Source: three-view drawing plus pictorial views. Frame: mm from the lowest corner of the part. A direction names the side the tool comes from. Coordinates: 2 decimals unless noted, no trailing zeros. Order: outer loops, then holes, each group sorted by start corner. A loop starts at its lowest first (then second) coordinate and runs counter-clockwise, first axis right, second up. Notation, with made-up numbers: M 88,77 L 102,77 A22 cw 102,95 Z; hole C -2,61.5 d1. An arc over 180 degrees is marked long. One line per question, with ' | ' between items.
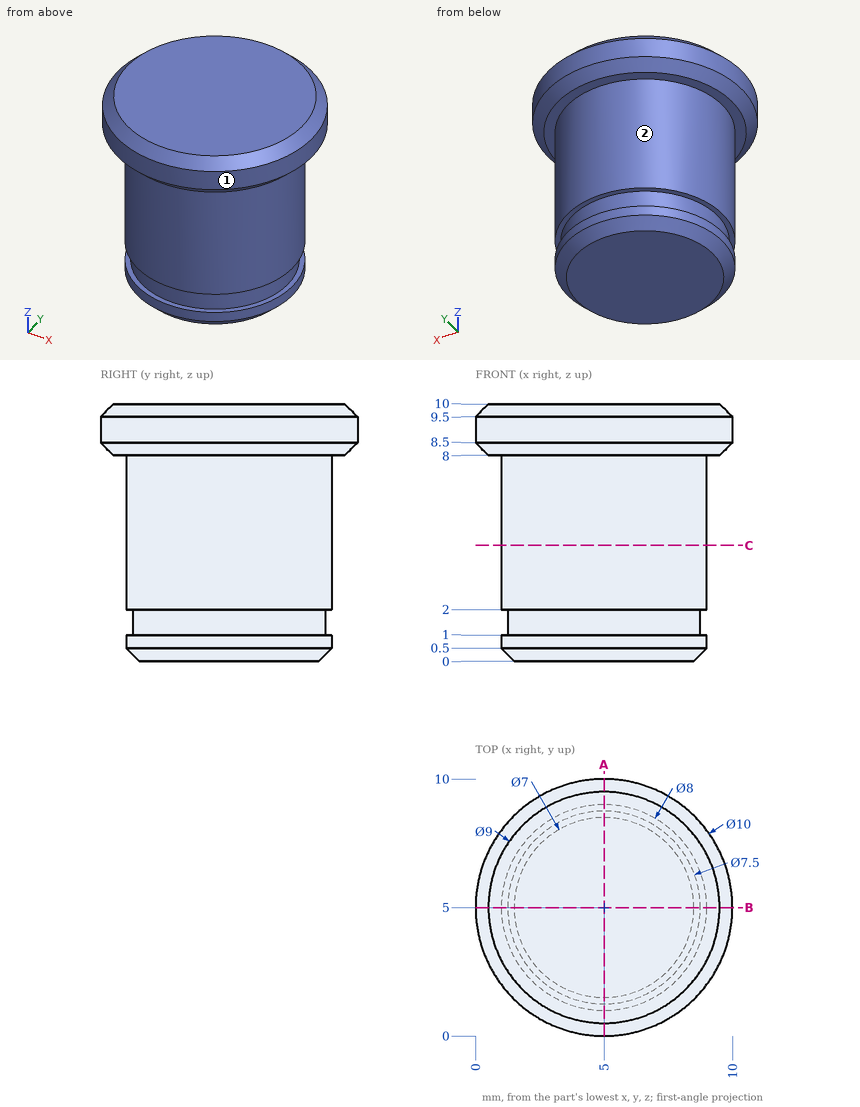
1. Pin query (flat end, axial travel): P1, Ø1.5, axis at y = 7.5, z = 6.5, coming from the +X side; P2, Ø3, axis at x = 2.5, z = 2, coming from the +Y side. Return the tip coordinate at first contact, or that it passes through.
Response values:
P1: stops at x = 8.6 | P2: stops at y = 8.87
2. Material intervals for line 1 (Z direction, x = 6.25, y = 9); line 2 (Y direction, x = 5, z = 6.75); line 3 (X direction, y = 5.5, z = 6), sorted ascending. Write a range as [from, to].
Response values:
line 1: z = [8, 10] | line 2: y = [1, 9] | line 3: x = [1.03, 8.97]
3. Access query for the marked faces 1 and 2. Directions: +Z, -Z, +X, -X, +Y, -Y. A direction counts if a zero-diameter tool reaches every point of the face in a straight line with its end or side. Return the directions, or none.
Response values:
face 1: +Z, -Z | face 2: -Z
4. Section C-C, the plane z = 4.5. Output: boundary loops of the cut face in (x, y), and give its area (3 significant figures).
Response values:
outline: C 5,5 d8 | area: 50.3 mm^2
5. Section A-A, the plane x = 5. Output: boundary loops of the cut face in (y, z).
Response values:
outline: M 0,8.5 L 0.5,8 L 1,8 L 1,2 L 1.25,2 L 1.25,1 L 1,1 L 1,0.5 L 1.5,0 L 8.5,0 L 9,0.5 L 9,1 L 8.75,1 L 8.75,2 L 9,2 L 9,8 L 9.5,8 L 10,8.5 L 10,9.5 L 9.5,10 L 0.5,10 L 0,9.5 Z
